from build123d import *

# Parameters (mm, degrees)
BASE_PLATE_DEPTH      = 10
FRONT_COLLAR_SKETCH_R = 19
FRONT_COLLAR_38_DEPTH = 7
FRONT_SHAFT_SKETCH_R  = 14
FRONT_SHAFT_28_DEPTH  = 35
REAR_COLLAR_SKETCH_R  = 19
REAR_COLLAR_38_DEPTH  = 7
REAR_SHAFT_SKETCH_R   = 14
REAR_SHAFT_28_DEPTH   = 35
REAR_BORE_SKETCH_R    = 7.5
REAR_BORE_15_DEPTH    = 35
FRONT_BORE_SKETCH_R   = 7.5
FRONT_BORE_15_DEPTH   = 35
END_HOLES_SKETCH_R    = 7.5
END_HOLES_2X_15_DEPTH = 10


with BuildPart() as part:
    # Base Plate Sketch → Base Plate (new body)
    with BuildSketch(Plane.XY):
        with BuildLine():
            Line((0, 22), (69, 22))
            Line((69, 22), (91, 22))
            Line((91, 22), (94, 19))
            Line((94, 19), (94, -19))
            Line((94, -19), (91, -22))
            Line((91, -22), (69, -22))
            Line((69, -22), (0, -22))
            ThreePointArc((0, -22), (-22, 0), (0, 22))
        make_face()
    extrude(amount=BASE_PLATE_DEPTH)

    # Front Collar Sketch → Front Collar Ø38 (add)
    with BuildSketch(Plane.XY.offset(10)):
        Circle(FRONT_COLLAR_SKETCH_R)
    extrude(amount=FRONT_COLLAR_38_DEPTH)

    # Front Shaft Sketch → Front Shaft Ø28 (add)
    with BuildSketch(Plane.XY.offset(17)):
        Circle(FRONT_SHAFT_SKETCH_R)
    extrude(amount=FRONT_SHAFT_28_DEPTH)

    # Rear Collar Sketch → Rear Collar Ø38 (add)
    with BuildSketch(Plane(origin=(0, 0, 0), x_dir=(-1, 0, 0), z_dir=(0, 0, -1))):
        with Locations(Location((-45.5, 0, 0), (0, 0, 180))):
            Circle(REAR_COLLAR_SKETCH_R)
    extrude(amount=REAR_COLLAR_38_DEPTH)

    # Rear Shaft Sketch → Rear Shaft Ø28 (add)
    with BuildSketch(Plane(origin=(0, 0, -7), x_dir=(-1, 0, 0), z_dir=(0, 0, -1))):
        with Locations((-45.5, 0)):
            Circle(REAR_SHAFT_SKETCH_R)
    extrude(amount=REAR_SHAFT_28_DEPTH)

    # Rear Bore Sketch → Rear Bore Ø15 (cut)
    with BuildSketch(Plane(origin=(0, 0, -42), x_dir=(-1, 0, 0), z_dir=(0, 0, -1))):
        with Locations((-45.5, 0)):
            Circle(REAR_BORE_SKETCH_R)
    extrude(amount=-REAR_BORE_15_DEPTH, mode=Mode.SUBTRACT)

    # Front Bore Sketch → Front Bore Ø15 (cut)
    with BuildSketch(Plane.XY.offset(52)):
        Circle(FRONT_BORE_SKETCH_R)
    extrude(amount=-FRONT_BORE_15_DEPTH, mode=Mode.SUBTRACT)

    # End Holes Sketch → End Holes 2xØ15 (cut)
    with BuildSketch(Plane.XY.offset(10)):
        with Locations((78.929188111, 12)):
            Circle(END_HOLES_SKETCH_R)
        with Locations((78.929188111, -12)):
            Circle(END_HOLES_SKETCH_R)
    extrude(amount=-END_HOLES_2X_15_DEPTH, mode=Mode.SUBTRACT)


solid = part.part
Design review of the part built by this model. Coordinates are the model's own, in mm. A direction names the side the tool comes from. Give positions to 0.01 mm unless a question says otherwise; leave off trailing zeros. Write each loop counter-clockwise with the first axis right and the second up, starting at its lowest first coordinate (ties: lowest second). Pieces come first, ordered by that corner, then holes. Notation, with made-up numbers: M -2,-25.75 L 9,-25.75 A26 ccw 9,1.25 Z; hole C 1,26.25 d1. An arc over 180 degrees is marked long. Return JSON: item names as keys, results as strings. Group by question number.
Item 1: Take a section at B-B (y = 12). Give the boundary of the cut face in (x, z), plus the area to 3 significant figures.
Item 2: Wall thickness on line 1 along Y through (x, z) = (45, -27); line 2 along Y through (x, z) = (76.5, 7.5); line 3 along Z through (x, y) = (36, -5.5): over which ranges is each line inside the solid? List them lowest first.
Item 3: Take a section at C-C (x = 45.5). Give the boundary of the cut face in (y, z), plus the area to 3 significant figures.
Item 4: The part is to be moulded in two halves that separate along Y. For faces 4 (the cylindrical face through (86.083, 14.253, 5.07)), 5 (the cylindrical face through (-22, 0, 5)), 6 (the flat face through (38, 13, -7)), 7 (the cylindrical face through (86.083, -9.747, 5.07)), say which applies: pulls with the +Y half, pulls with the -Y half, needs draft (parallel to the pull), parting line crosses it, or undercut.
Item 5: Clearance check with flat-ended pins moving along their axes: pin 1 Ø4 at (x, y) = (11, 2) entering from -Z; pin 2 Ø12 at (x, y) = (45, -1) entering from -Z; pin 3 Ø19.5 at (x, y) = (45.5, 0) entering from -Z; pin 4 Ø10 at (x, y) = (57.5, -17) entering from +Z. State where each tip first meets the part, or that it passes through.
Item 6: Take a section at D-D (z = -30). Give the boundary of the cut face in (x, y), plus the area to 3 significant figures.
Item 7: Tool access review of faces 1 (the cylindrical face through (38.346, 2.253, -24.745)), 2 (the cylindrical face through (-7.493, 0.33, 34.745)), 3 (the flat face through (6, -6, 52)): name each direction out of +Z, -Z, +X, -X, +Y, -Y from which nothing blocks a thin tool from reaching the whole face with its end or side.
Item 8: Take a section at A-A (x = 76.5). Give the boundary of the cut face in (y, z), plus the area to 3 significant figures.
Return value:
{
 "1": {"outline": "M -18.44,0 L 30.77,0 L 30.77,-7 L 38.29,-7 L 38.29,-42 L 52.71,-42 L 52.71,-7 L 60.23,-7 L 60.23,0 L 71.43,0 L 71.43,10 L 14.73,10 L 14.73,17 L 7.21,17 L 7.21,52 L -7.21,52 L -7.21,17 L -14.73,17 L -14.73,10 L -18.44,10 Z; M 86.43,0 L 94,0 L 94,10 L 86.43,10 Z", "area": "2,400 mm2"},
 "2": {"line 1": "y = -13.99 to -7.48, 7.48 to 13.99", "line 2": "y = -22 to -19.1, -4.9 to 4.9, 19.1 to 22", "line 3": "z = -42 to 10"},
 "3": {"outline": "M -22,0 L -19,0 L -19,-7 L -14,-7 L -14,-42 L -7.5,-42 L -7.5,-7 L 7.5,-7 L 7.5,-42 L 14,-42 L 14,-7 L 19,-7 L 19,0 L 22,0 L 22,10 L -22,10 Z", "area": "1,160 mm2"},
 "4": {"face 4": "undercut", "face 5": "parting line crosses it", "face 6": "needs draft", "face 7": "undercut"},
 "5": {"pin 1": "stops at z = 0", "pin 2": "stops at z = -7", "pin 3": "stops at z = -42", "pin 4": "stops at z = 10"},
 "6": {"outline": "C 45.5,0 d28; hole C 45.5,0 d15", "area": "439 mm2"},
 "7": {"face 1": "-Z", "face 2": "+Z", "face 3": "+Z, +X, -X, +Y, -Y"},
 "8": {"outline": "M -22,0 L -19.1,0 L -19.1,10 L -22,10 Z; M -4.9,0 L 4.9,0 L 4.9,10 L -4.9,10 Z; M 19.1,0 L 22,0 L 22,10 L 19.1,10 Z", "area": "156 mm2"}
}
